The figure shows three views and two pictorial views of one solid part (mm, origin at its lowest corner). Answer the questions. Give positions to 0.01 mm unless a question says otherwise; leave off trailing zeros. Loops run counter-clockwise (first coordinate to the right, second up) from the corner with the lowest first, then second, coordinate; pieces in that order, holes last. Notation, with made-up numbers: (-35.5, 79.25) - (-2.5, 79.25) arc R24 ccw to (-2.5, 111.25) - close; hole circle Ø4 at (45.5, -27). An arc over 180 degrees is marked (long way). Use a Markdown table: item, result. Add a question column.
Item 1: A cutting plane is placed at C-C (z = 198). Determine the outline of the cut face in (x, y), plus the area to 4 significant figures.
Item 2: For a pull along Z with two mould halves and no side action, classify the marked faces 1, 2 and 3 as +Z half, -Z half, draft (parallel to the pull), parting line (faces both ways), or undercut.
Item 3: This flat-tipped pin is pushed along its axis until it touches: P1, Ø1, axis at x = 122, y = 10, coming from the -Z side. Where does it stop, or does it pass through?
Item 4: A cutting plane is placed at B-B (y = 15). Determine the outline of the cut face in (x, z).
Item 5: A cutting plane is placed at D-D (x = 187.5). Determine the outline of the cut face in (y, z).
Item 6: A cutting plane is placed at A-A (z = 120). Determine the outline of the cut face in (x, y).
Item 7: Consider probe 1 along Z at (x, y) = (192, 16); probe 2 along X at (y, z) = (35, 120); probe 3 along X at (y, z) = (4.5, 198). Determine where each line is inside the solid, lowest interval first. Write a range as [from, to].
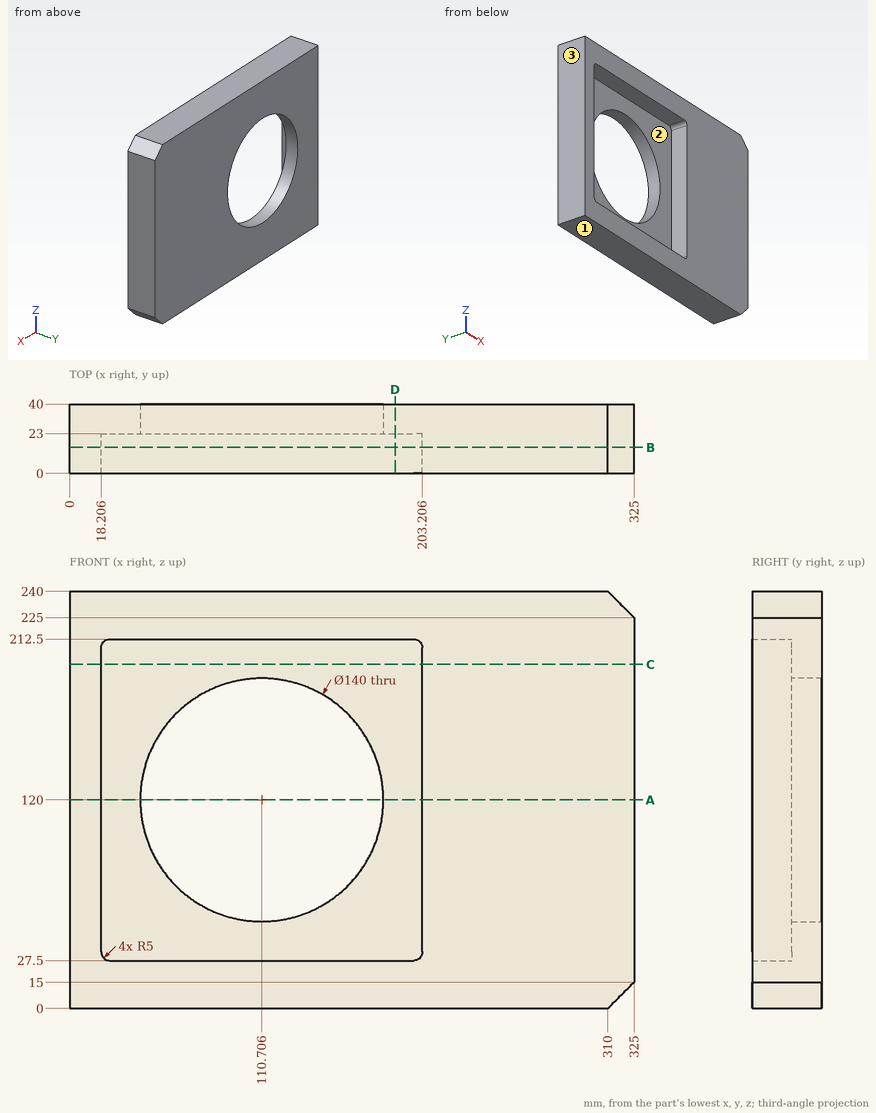
Geometry says:
| question | item | result |
|---|---|---|
| 1 | outline | (0, 0) - (18.21, 0) - (18.21, 23) - (203.21, 23) - (203.21, 0) - (325, 0) - (325, 40) - (0, 40) - close |
| 1 | area | 8,745 mm² |
| 2 | face 1 | -Z half |
| 2 | face 2 | undercut |
| 2 | face 3 | draft |
| 3 | P1 | z = 0 |
| 4 | outline | (0, 0) - (310, 0) - (325, 15) - (325, 225) - (310, 240) - (0, 240) - close; hole (18.21, 32.5) arc R5 ccw to (23.21, 27.5) - (198.21, 27.5) arc R5 ccw to (203.21, 32.5) - (203.21, 207.5) arc R5 ccw to (198.21, 212.5) - (23.21, 212.5) arc R5 ccw to (18.21, 207.5) - close |
| 5 | outline | (0, 0) - (40, 0) - (40, 240) - (0, 240) - (0, 212.5) - (23, 212.5) - (23, 27.5) - (0, 27.5) - close |
| 6 | outline | (0, 0) - (18.21, 0) - (18.21, 23) - (40.71, 23) - (40.71, 40) - (0, 40) - close; (180.71, 23) - (203.21, 23) - (203.21, 0) - (325, 0) - (325, 40) - (180.71, 40) - close |
| 7 | probe 1 | [0, 27.5], [212.5, 240] |
| 7 | probe 2 | [0, 40.71], [180.71, 325] |
| 7 | probe 3 | [0, 18.21], [203.21, 325] |
